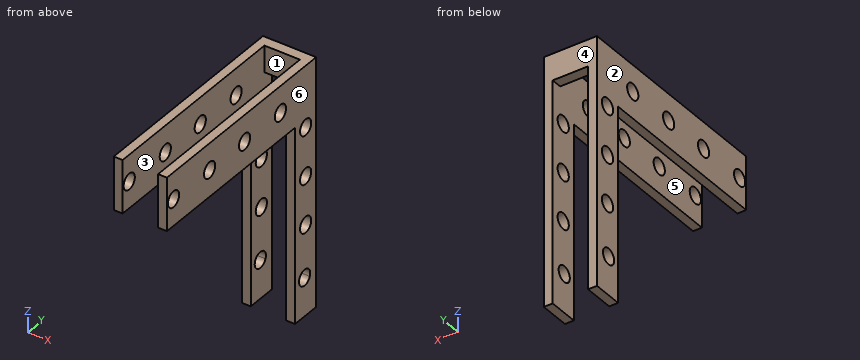
```python
from build123d import *

# Parameters (mm, degrees)
SKETCH1_W             = 50
SKETCH1_H             = 300
BOSS_EXTRUDE1_DEPTH   = 1200
BOSS_EXTRUDE1_2_DEPTH = 1200
BOSS_EXTRUDE2_REACH   = 1236.909
SKETCH2_W             = 300
SKETCH2_H             = 60
SKETCH3_R             = 45
CUT_EXTRUDE1_DEPTH    = 900
SKETCH5_W             = 50
SKETCH5_H             = 170
BOSS_EXTRUDE3_DEPTH   = 900
SKETCH7_R             = 45
CUT_EXTRUDE2_DEPTH    = 900
SKETCH8_W             = 200
SKETCH8_H             = 150
CUT_EXTRUDE3_DEPTH    = 137
SKETCH9_R             = 45.000000002
CUT_EXTRUDE4_DEPTH    = 408
SKETCH10_R            = 45
CUT_EXTRUDE5_DEPTH    = 997
BOSS_EXTRUDE4_START   = -50
BOSS_EXTRUDE4_DEPTH   = 50
BOSS_EXTRUDE5_DEPTH   = 50


with BuildPart() as part:
    # Sketch1 → Boss-Extrude1 (new body)
    with BuildSketch(Plane(origin=(0, 0, 0), x_dir=(1, 0, 0), z_dir=(0, 1, 0))):
        with Locations((125, 0)):
            Rectangle(SKETCH1_W, SKETCH1_H)
    extrude(amount=BOSS_EXTRUDE1_DEPTH)

    # Sketch2 → Boss-Extrude2 (add, up to next)
    with BuildSketch(Plane(origin=(-100, 0, 0), x_dir=(0, 0, -1), z_dir=(1, 0, 0)), mode=Mode.PRIVATE) as boss_extrude2_sk1:
        with Locations((0, 1170)):
            Rectangle(SKETCH2_W, SKETCH2_H)
    boss_extrude2_tool1 = extrude(boss_extrude2_sk1.sketch, amount=BOSS_EXTRUDE2_REACH, mode=Mode.PRIVATE) - part.part


with BuildPart() as body_2:
    # Sketch1 → Boss-Extrude1 2 (new body)
    with BuildSketch(Plane(origin=(0, 0, 0), x_dir=(1, 0, 0), z_dir=(0, 1, 0))):
        with Locations((-125, 0)):
            Rectangle(SKETCH1_W, SKETCH1_H)
    extrude(amount=BOSS_EXTRUDE1_2_DEPTH)


with BuildPart() as part_1:
    add(part.part)

    add(body_2.part)  # Boss-Extrude2 merges body 2
    add(boss_extrude2_tool1.solids().sort_by_distance((-100, 1170, 0))[0])

    # Sketch3 → Cut-Extrude1 (cut)
    with BuildSketch(Plane(origin=(150, 0, 0), x_dir=(0, 0, -1), z_dir=(1, 0, 0))):
        with Locations((0, 624)):
            Circle(SKETCH3_R)
        with Locations((0, 343)):
            Circle(SKETCH3_R)
        with Locations((0, 53)):
            Circle(SKETCH3_R)
    extrude(amount=-CUT_EXTRUDE1_DEPTH, mode=Mode.SUBTRACT)

    # Sketch5 → Boss-Extrude3 (add)
    with BuildSketch(Plane(origin=(0, 0, -150), x_dir=(-1, 0, 0), z_dir=(0, 0, -1))):
        with Locations((-125, 1115)):
            Rectangle(SKETCH5_W, SKETCH5_H)
        with Locations((125, 1115)):
            Rectangle(SKETCH5_W, SKETCH5_H)
    extrude(amount=BOSS_EXTRUDE3_DEPTH)

    # Sketch7 → Cut-Extrude2 (cut)
    with BuildSketch(Plane(origin=(150, 0, 0), x_dir=(0, 0, -1), z_dir=(1, 0, 0))):
        with Locations((468.812102097, 1115)):
            Circle(SKETCH7_R)
        with Locations((741.013548247, 1115)):
            Circle(SKETCH7_R)
        with Locations((195.161471607, 1115)):
            Circle(SKETCH7_R)
    extrude(amount=-CUT_EXTRUDE2_DEPTH, mode=Mode.SUBTRACT)

    # Sketch8 → Cut-Extrude3 (cut)
    with BuildSketch(Plane(origin=(0, 1200, 0), x_dir=(1, 0, 0), z_dir=(0, 1, 0))):
        with Locations((0, 75)):
            Rectangle(SKETCH8_W, SKETCH8_H)
    extrude(amount=-CUT_EXTRUDE3_DEPTH, mode=Mode.SUBTRACT)

    # Sketch9 → Cut-Extrude4 (cut)
    with BuildSketch(Plane(origin=(150, 0, 0), x_dir=(0, 0, -1), z_dir=(1, 0, 0))):
        with Locations((1032.951729484, 1106.805056962)):
            Circle(SKETCH9_R)
    extrude(amount=-CUT_EXTRUDE4_DEPTH, mode=Mode.SUBTRACT)

    # Sketch10 → Cut-Extrude5 (cut)
    with BuildSketch(Plane.ZY.offset(150)):
        with Locations((0, 912.304081816)):
            Circle(SKETCH10_R)
    extrude(amount=-CUT_EXTRUDE5_DEPTH, mode=Mode.SUBTRACT)

    # Sketch12 → Boss-Extrude4 (add)
    with BuildSketch(Plane.ZY.offset(150).offset(BOSS_EXTRUDE4_START)):
        with BuildLine():
            Line((-1050, 1200), (-1250, 1200))
            Line((-1250, 1200), (-1250, 1030))
            Line((-1250, 1030), (-1050, 1030))
            Line((-1050, 1030), (-1050, 1065.159451282))
            ThreePointArc((-1050, 1065.159451282), (-1077.951729484, 1106.805056962), (-1050, 1148.450662641))
            Line((-1050, 1148.450662641), (-1050, 1200))
        make_face()
    extrude(amount=BOSS_EXTRUDE4_DEPTH)

    # Sketch13 → Boss-Extrude5 (add)
    with BuildSketch(Plane(origin=(150, 0, 0), x_dir=(0, 0, -1), z_dir=(1, 0, 0))):
        with BuildLine():
            Line((1250, 1200), (1050, 1200))
            Line((1050, 1200), (1050, 1148.450662641))
            ThreePointArc((1050, 1148.450662641), (1077.951729484, 1106.805056962), (1050, 1065.159451282))
            Line((1050, 1065.159451282), (1050, 1030))
            Line((1050, 1030), (1250, 1030))
            Line((1250, 1030), (1250, 1200))
        make_face()
    extrude(amount=-BOSS_EXTRUDE5_DEPTH)


solid = part_1.part
```
Input: part model. Units: mm. Frame: model coordinates. Face numbers are marked on the shaded views. A direction names the side the tool comes from. Coordinates: 2 decimals unless noted, no trailing zeros. Write each loop counter-clockwise with the first axis right and the second up, starting at its lowest first coordinate (ties: lowest second). Pieces come first, ordered by that corner, then holes. Notation, with made-up numbers: (48, 72) - (87, 72) arc R15 cw to (87, 85) - close; hole circle Ø8 at (87, 29). An arc over 180 degrees is marked (long way). Put each result on its own line as item: value. Start each with the question number.
1) Mould query, pull axis X, two halves, no side actions, for the marked faces 4, 5 and 6. Classes: pulls with the +X half, pulls with the -X half, needs draft (parallel to the pull), parting line crosses it, or undercut.
2) Contact query for flat-ended pins moving along their axis: pin 1 (15 mm diameter, centred on x = 127, y = 482, fed in from -Z); pin 2 (25 mm diameter, centred on x = 120.5, z = -937.5, fed in from -Y). Output: stop coordinate, or through.
3) Ray query, L1, parallel to Y at x = 132, z = 0; L2, parallel to X at y = 167, z = -7; L3, parallel to Y at x = 109.5, z = 12.5. Return the intervals inside material, ascending.
4) Cut plane A-A (z = -927.5). Return the cut outline in (x, y).
5) Cut plane B-B (y = 782). Return the cut outline in (x, z).
6) Cut plane C-C (y = 624). Return the cut outline in (x, z), plus the area to 3 significant figures.
7) Cut plane D-D (x = -127). State how many separate pieces and enclosed holes the cut face has, plus the area to 3 significant figures.
8) Reachability of the marked faces 1, 2 and 3 from +Z, -Z, +X, -X, +Y, -Y: full face, straight path, thin tool, end or side. Return the list, or none.
Resolved:
1. face 4: needs draft
1. face 5: undercut
1. face 6: pulls with the +X half
2. pin 1: stops at z = -150
2. pin 2: stops at y = 1030
3. L1: y = 0 to 8, 98 to 298, 388 to 579, 669 to 867.3, 957.3 to 1200
3. L2: x = -150 to -100, 100 to 150
3. L3: y = 0 to 9.77, 96.23 to 299.77, 386.23 to 580.77, 667.23 to 869.08, 955.53 to 1200
4. outline: (-150, 1030) - (-100, 1030) - (-100, 1200) - (-150, 1200) - close; (100, 1030) - (150, 1030) - (150, 1200) - (100, 1200) - close
5. outline: (-150, -150) - (-100, -150) - (-100, 150) - (-150, 150) - close; (100, -150) - (150, -150) - (150, 150) - (100, 150) - close
6. outline: (-150, -150) - (-100, -150) - (-100, -45) - (-150, -45) - close; (-150, 45) - (-100, 45) - (-100, 150) - (-150, 150) - close; (100, -150) - (150, -150) - (150, -45) - (100, -45) - close; (100, 45) - (150, 45) - (150, 150) - (100, 150) - close
6. area: 21,000 mm2
7. separate pieces: 1
7. enclosed holes: 8
7. area: 496,000 mm2
8. face 1: +Z, -Z, -Y
8. face 2: +Z, -Z, -X, +Y, -Y
8. face 3: -Z, -Y
